Source: CAD feature listing. Evaluate the final solid. Frame: model axes, mm. A direction names the side the tool comes from. Give positions to 0.01 mm unless a question says otherwise; leave off trailing zeros. Order: outer loops, then holes, each group sorted by start corner. A loop starts at its lowest first (then second) coordinate and runs counter-clockwise, first axis right, second up. Notation, with made-up numbers: M -34.75,25.5 L 1.25,25.5 A19 cw 1.25,33.5 Z; hole C -36,63 d9. An arc over 180 degrees is marked long. Answer as a JSON object with one key per item and string values. Group by question number.
1. Section query B-B (z = 419). Output: boundary loops of the cut face in (x, y), plus the area to 3 significant figures.
2. Pin query (flat end, axial travel): P1, Ø1.3, axis at y = 16, z = -2.5, coming from the +X side; P2, Ø1.7, axis at y = 9, z = 446.5, coming from the +X side; P3, Ø1.1, axis at y = 9, z = 449, coming from the -X side. Return the tip coordinate at first contact, or that it passes through.
3. Section query A-A (y = 0). Output: boundary loops of the cut face in (x, z).
4. Material intervals for L1, parallel to Z at x = -10, y = -3.5; L2, parallel to Z at x = 11, y = -6; L3, parallel to Y at x = 0.5, z = 175.5, sorted ascending. Write a range as [from, to].
5. Set-up query: faces 1 (the cylindrical face through (10.316, 7.91, 190.91)), 2 (the flat face through (-7, 8, 255)), 3 (the flat face through (0, 13, -5)). Return all of +Z, -Z, +X, -X, +Y, -Y with unobstructed straight access to the full face (end or side cutting, diameter ignored); none if empty.
6. Pull-direction query (Z, two-part tool) for faces 4 (the flat face through (6, 3, 125)), 5 (the cylindrical face through (10.316, 7.91, 360.91)), 6 (the flat face through (-7, 8, 425)); classes: +Z half, -Z half, draft (parallel to the pull), parting line (faces both ways), or undercut.
from build123d import *
from build123d.topology import SkipClean

# Parameters (mm, degrees)
SKETCH1_R           = 18
BOSS_EXTRUDE2_DEPTH = 25
SKETCH6_R           = 12
BOSS_EXTRUDE6_DEPTH = 60
SKETCH7_R           = 6
BOSS_EXTRUDE7_DEPTH = 30
CUT_EXTRUDE3_DEPTH  = 10
CUT_EXTRUDE4_DEPTH  = 5
CUT_EXTRUDE5_DEPTH  = 2.5
CUT_EXTRUDE6_DEPTH  = 2.5


with BuildPart() as part:
    # Sketch1 → Boss-Extrude2 (new, symmetric)
    with BuildSketch(Plane.XY):
        Circle(SKETCH1_R)
    extrude(amount=BOSS_EXTRUDE2_DEPTH, both=True)

    # Sketch6 → Boss-Extrude6 (add)
    with BuildSketch(Plane.XY.offset(25)):
        Circle(SKETCH6_R)
    extrude(amount=BOSS_EXTRUDE6_DEPTH)

    # Sketch7 → Boss-Extrude7 (add)
    with BuildSketch(Plane.XY.offset(85)):
        Circle(SKETCH7_R)
    extrude(amount=BOSS_EXTRUDE7_DEPTH)

    # Sketch11 → Cut-Extrude3 (cut)
    with BuildSketch(Plane(origin=(0, 13, 0), x_dir=(-1, 0, 0), z_dir=(0, 1, 0))):
        with BuildLine():
            Line((-5, 0), (-5, -10))
            ThreePointArc((-5, -10), (0, -15), (5, -10))
            Line((5, -10), (5, 0))
            ThreePointArc((5, 0), (0, 5), (-5, 0))
        make_face()
    extrude(amount=CUT_EXTRUDE3_DEPTH, mode=Mode.SUBTRACT)

    # Sketch12 → Cut-Extrude4 (cut)
    with BuildSketch(Plane(origin=(0, 5, 0), x_dir=(-1, 0, 0), z_dir=(0, 1, 0))):
        with BuildLine():
            Line((-1.4, 110.5), (-1.4, 93.3))
            ThreePointArc((-1.4, 93.3), (0, 91.9), (1.4, 93.3))
            Line((1.4, 93.3), (1.4, 110.5))
            ThreePointArc((1.4, 110.5), (0, 111.9), (-1.4, 110.5))
        make_face()
    extrude(amount=CUT_EXTRUDE4_DEPTH, mode=Mode.SUBTRACT)

    # Sketch13 → Revolve1 (revolve)
    with SkipClean():  # the faces are left unmerged after this step: merging them gives an invalid solid
        with BuildSketch(Plane(origin=(0, 0, 0), x_dir=(1, 0, 0), z_dir=(0, 1, 0))):
            Polygon((0, -465), (0, -115), (-6, -115), (-6, -125), (-13, -125), (-13, -255), (-10, -255), (-10, -295), (-13, -295), (-13, -425), (-10, -425), (-10, -465), align=None)
        revolve(axis=Axis((0, 0, 75.161405529), (0, 0, 1)))

    # Sketch16 → Cut-Extrude5 (cut)
    with SkipClean():  # the faces are left unmerged after this step: merging them gives an invalid solid
        with BuildSketch(Plane(origin=(0, 10, 0), x_dir=(1, 0, 0), z_dir=(0, 1, 0))):
            with BuildLine():
                Line((2.5, -265), (2.5, -285))
                ThreePointArc((2.5, -285), (0, -287.5), (-2.5, -285))
                Line((-2.5, -285), (-2.5, -265))
                ThreePointArc((-2.5, -265), (0, -262.5), (2.5, -265))
            make_face()
        extrude(amount=-CUT_EXTRUDE5_DEPTH, mode=Mode.SUBTRACT)

    # Sketch17 → Cut-Extrude6 (cut)
    with SkipClean():  # the faces are left unmerged after this step: merging them gives an invalid solid
        with BuildSketch(Plane(origin=(0, 10, 0), x_dir=(1, 0, 0), z_dir=(0, 1, 0))):
            with BuildLine():
                Line((2.5, -435), (2.5, -455))
                ThreePointArc((2.5, -455), (0, -457.5), (-2.5, -455))
                Line((-2.5, -455), (-2.5, -435))
                ThreePointArc((-2.5, -435), (0, -432.5), (2.5, -435))
            make_face()
        extrude(amount=-CUT_EXTRUDE6_DEPTH, mode=Mode.SUBTRACT)


solid = part.part
Answer sheet:
{
 "1": {"outline": "C 0,0 d26", "area": "531 mm^2"},
 "2": {"P1": "x = 9.4", "P2": "x = 5.79", "P3": "x = -5.35"},
 "3": {"outline": "M -18,-25 L 18,-25 L 18,25 L 12,25 L 12,85 L 6,85 L 6,125 L 13,125 L 13,255 L 10,255 L 10,295 L 13,295 L 13,425 L 10,425 L 10,465 L -10,465 L -10,425 L -13,425 L -13,295 L -10,295 L -10,255 L -13,255 L -13,125 L -6,125 L -6,85 L -12,85 L -12,25 L -18,25 Z"},
 "4": {"L1": "[-25, 85], [125, 255], [295, 425]", "L2": "[-25, 25], [125, 255], [295, 425]", "L3": "[-12.99, 12.99]"},
 "5": {"face 1": "+Z", "face 2": "none", "face 3": "+Y"},
 "6": {"face 4": "undercut", "face 5": "draft", "face 6": "+Z half"}
}
